Geometry check sheet. Reference: drawing and pictorial views, mm from the part's lowest x, y, z. Round coordinates to 2 decimals unless told otherwise and drop trailing zeros. Write each loop counter-clockwise with the first axis right and the second up, starting at its lowest first coordinate (ties: lowest second). Pieces come first, ordered by that corner, then holes. Notation, with made-up numbers: (1, -25.75) - (28, -25.75) arc R23 ccw to (28, 9.25) - close; hole circle Ø9 at (80, 0.5). An arc over 180 degrees is marked (long way). Use one line per item in the form item = value. Start each with the question number.
1) Gauge pin test, flat ends, axial feed: P1, Ø6, axis at x = 3, y = 29, coming from the +Z side; P2, Ø1.5, axis at x = 16.5, y = 16.5, coming from the +Z side; P3, Ø1, axis at x = 16, y = 20.5, coming from the -Z side. Record the tip position at first contact, or that the pin passes through.
2) Scan lines: probe 1 along X at (y, z) = (9, 1); probe 2 along Z at (x, y) = (1, 31.5); probe 3 along X at (y, z) = (2.5, 9.5). Record each from-to range of solid material in increasing order.
3) Section check A-A (y = 21.5). Record the boundary of the cut face in (x, z).
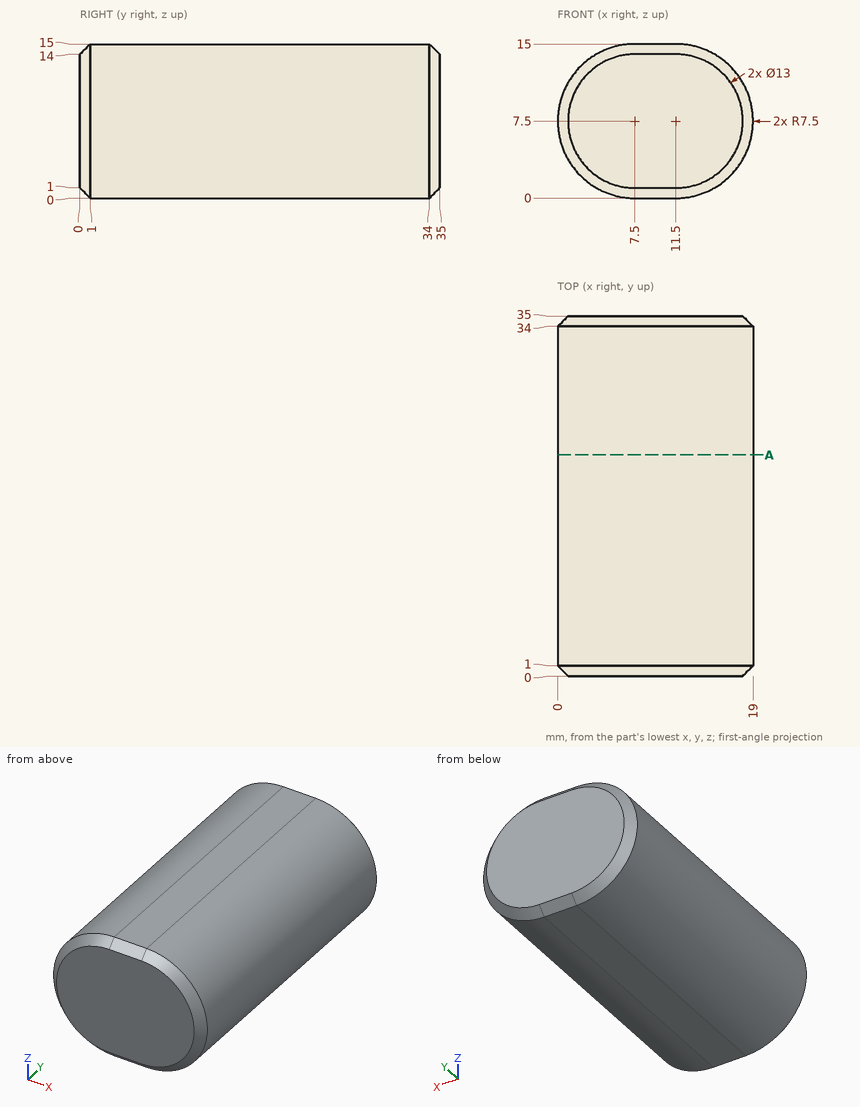
Results are:
q1.P1 = 14.85
q1.P2 = 13.68
q1.P3 = 1.16
q2.probe_1 = 3.76 to 15.24
q2.probe_2 = 3.76 to 11.24
q2.probe_3 = 0.27 to 18.73
q3.outline = (7.5, 0) - (11.5, 0) arc R7.5 ccw to (11.5, 15) - (7.5, 15) arc R7.5 ccw to start
